Verification items for the finished model (mm, model axes). Round coordinates to 2 decimals unless told otherwise and drop trailing zeros. Order: outer loops, then holes, each group sorted by start corner. A loop starts at its lowest first (then second) coordinate and runs counter-clockwise, first axis right, second up. Notation, with made-up numbers: (-24, 0) -> (5, 0) arc R19 cw to (5, 30) -> close; hole circle Ø4 at (61, -23.75). An arc over 180 degrees is marked (long way). Put each result on its own line as item: value.
from build123d import *

# Parameters (mm, degrees)
SKETCH_1_W          = 24
SKETCH_1_H          = 52
EXTRUDE_1_DEPTH     = 4
SKETCH_2_R          = 3.2
CUT_EXTRUDE_1_DEPTH = 14


with BuildPart() as part:
    # 草图1 → 凸台-拉伸1 (new, symmetric)
    with BuildSketch(Plane.XY):
        Rectangle(SKETCH_1_W, SKETCH_1_H)
    extrude(amount=EXTRUDE_1_DEPTH, both=True)

    # 草图2 → 切除-拉伸1 (cut, symmetric)
    with BuildSketch(Plane.XY):
        with Locations((-5, -18)):
            Circle(SKETCH_2_R)
        with Locations((5, 18)):
            Circle(SKETCH_2_R)
    extrude(amount=CUT_EXTRUDE_1_DEPTH, both=True, mode=Mode.SUBTRACT)


solid = part.part
Item 1: Release check for a two-part mould opening along Y. For faces 1 (the flat face through (0, 0, 4)), 2 (the cylindrical face through (-5.694, -21.124, 0.056)), 3 (the flat face through (0, 26, 0)), 4 (the cylindrical face through (4.306, 14.876, 0.056)) record: +Y half, -Y half, draft (parallel to the pull), parting line (faces both ways), or undercut.
Check sheet entries:
face 1: draft
face 2: undercut
face 3: +Y half
face 4: undercut
Item 2: Section check C-C on z = 3. Record the boundary of the cut face in (x, y), then the cut area to 3 significant figures.
Check sheet entries:
outline: (-12, -26) -> (12, -26) -> (12, 26) -> (-12, 26) -> close; hole circle Ø6.4 at (-5, -18); hole circle Ø6.4 at (5, 18)
area: 1,180 mm^2
Item 3: Section check A-A on y = -18. Record the boundary of the cut face in (x, z), then the cut area to 3 significant figures.
Check sheet entries:
outline: (-12, -4) -> (-8.2, -4) -> (-8.2, 4) -> (-12, 4) -> close; (-1.8, -4) -> (12, -4) -> (12, 4) -> (-1.8, 4) -> close
area: 141 mm^2
Item 4: Material ranges on L1, parallel to Y at x = 5, z = 2.75; L2, parallel to Y at x = -4.75, z = 1.25; L3, parallel to X at y = -18, z = -0.5, recorded low to high. Write a range as [from, to].
Check sheet entries:
L1: y = [-26, 14.8], [21.2, 26]
L2: y = [-26, -21.19], [-14.81, 26]
L3: x = [-12, -8.2], [-1.8, 12]
Item 5: Section check B-B on x = -5. Record the boundary of the cut face in (y, z).
Check sheet entries:
outline: (-26, -4) -> (-21.2, -4) -> (-21.2, 4) -> (-26, 4) -> close; (-14.8, -4) -> (26, -4) -> (26, 4) -> (-14.8, 4) -> close
Item 6: Gauge pin test, flat end, axial feed: pin 1 Ø1 at (x, y) = (-6, -19.5) entering from -Z. Record the tip position at first contact, or that the pin passes through.
Check sheet entries:
pin 1: passes through
